Answer from the drawing. Dimensions are ordinates in mm from the lowest x, y and z of the part. Give positions to 0.01 mm unless a question says otherwise; leave off trailing zeros. Write each loop counter-clockwise with the first axis right and the second up, starting at its lowest first coordinate (ties: lowest second). Pieces come first, ordered by that corner, then holes.
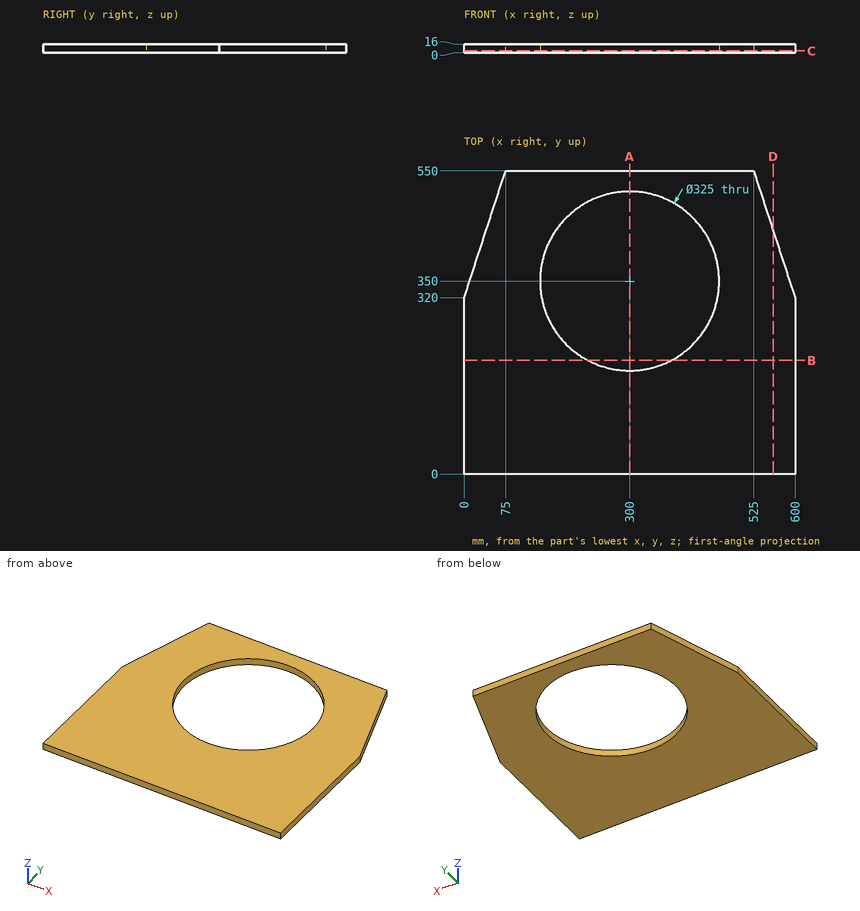
Item 1: A cutting plane is placed at D-D, the plane x = 560.5. Give the vertices of the cut face in (y, z), plus the area to 3 significant figures.
Conclusion:
outline: (0, 0) - (441.13, 0) - (441.13, 16) - (0, 16) - close
area: 7,060 mm2
Item 2: A cutting plane is placed at A-A, the plane x = 300. Give the vertices of the cut face in (y, z).
Conclusion:
outline: (0, 0) - (187.5, 0) - (187.5, 16) - (0, 16) - close; (512.5, 0) - (550, 0) - (550, 16) - (512.5, 16) - close
Item 3: Consider probe 1 along Y at (x, z) = (300, 11.75); probe 2 along X at (y, z) = (353.5, 8.5); probe 3 along X at (y, z) = (367.5, 12.5). Determine where each line is inside the solid, lowest interval first.
Conclusion:
probe 1: y = 0 to 187.5, 512.5 to 550
probe 2: x = 10.92 to 137.54, 462.46 to 589.08
probe 3: x = 15.49 to 138.45, 461.55 to 584.51
Item 4: A cutting plane is placed at C-C, the plane z = 3.5. Give the vertices of the cut face in (x, y).
Conclusion:
outline: (0, 0) - (600, 0) - (600, 320) - (525, 550) - (75, 550) - (0, 320) - close; hole circle Ø325 at (300, 350)
Item 5: A cutting plane is placed at B-B, the plane y = 206. Give the vertices of the cut face in (x, z).
Conclusion:
outline: (0, 0) - (224.7, 0) - (224.7, 16) - (0, 16) - close; (375.3, 0) - (600, 0) - (600, 16) - (375.3, 16) - close
